```python
from build123d import *

# Parameters (mm, degrees)
BASE_BLOCK_SKETCH_W       = 50
BASE_BLOCK_SKETCH_H       = 30
BASE_BLOCK_50X30X25_DEPTH = 25
CORNER_STEP_5MM_DEPTH     = 5
LOWER_PLATE_SKETCH_W      = 19.888158271
LOWER_PLATE_SKETCH_H      = 16.417205811
LOWER_PLATE_5MM_DEPTH     = 5
LEG_SKETCH_W              = 5
LEG_SKETCH_H              = 16.417205811
LEG_15MM_DEPTH            = 15
TAPERED_WEB_16_5MM_DEPTH  = 16.5


with BuildPart() as part:
    # Base Block Sketch → Base Block 50x30x25 (new body)
    with BuildSketch(Plane(origin=(0, 0, 0), x_dir=(1, 0, 0), z_dir=(0, 1, 0))):
        with Locations((25, 15)):
            Rectangle(BASE_BLOCK_SKETCH_W, BASE_BLOCK_SKETCH_H)
    extrude(amount=BASE_BLOCK_50X30X25_DEPTH)

    # Corner Step Sketch → Corner Step 5mm (add)
    with BuildSketch(Plane(origin=(0, 0, 0), x_dir=(1, 0, 0), z_dir=(0, 1, 0))):
        Polygon((0, 30), (0, 40), (10, 40), (10, 35), (40, 35), (40, 40), (50, 40), (50, 30), (50, 0), (0, 0), align=None)
    extrude(amount=CORNER_STEP_5MM_DEPTH)

    # Lower Plate Sketch → Lower Plate 5mm (add)
    with BuildSketch(Plane.XZ):
        Polygon((6.770734002, 0), (0, 0), (0, -16.417205811), (6.770734002, -16.417205811), (20.078313967, -16.417205811), (20.078313967, 0), align=None)
        with Locations((40.055920865, -8.208602906)):
            Rectangle(LOWER_PLATE_SKETCH_W, LOWER_PLATE_SKETCH_H)
    extrude(amount=LOWER_PLATE_5MM_DEPTH)

    # Leg Sketch → Leg 15mm (add)
    with BuildSketch(Plane(origin=(0, -5, 0), x_dir=(-1, 0, 0), z_dir=(0, -1, 0))):
        with Locations((-2.5, 8.208602906)):
            Rectangle(LEG_SKETCH_W, LEG_SKETCH_H)
        with Locations((-47.5, 8.208602906)):
            Rectangle(LEG_SKETCH_W, LEG_SKETCH_H)
    extrude(amount=LEG_15MM_DEPTH)

    # Tapered Web Sketch → Tapered Web 16.5mm (add)
    with BuildSketch(Plane.XY):
        Polygon((30.111841729, -5), (45, -20), (45, -5), align=None)
        Polygon((5, -5), (5, -20), (20, -5), align=None)
    extrude(amount=-TAPERED_WEB_16_5MM_DEPTH)


solid = part.part
```
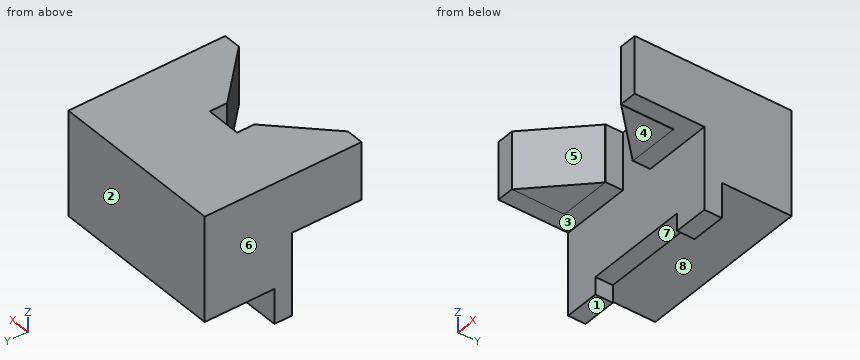
Input: part model. Units: mm. Frame: model coordinates. Face numbers are marked on the shaded views. A direction names the side the tool comes from. Give positions to 0.01 mm unless a question says otherwise; leave off trailing zeros. Write each loop counter-clockwise with the first axis right and the second up, starting at its lowest first coordinate (ties: lowest second). Pieces come first, ordered by that corner, then holes. Notation, with made-up numbers: (-12.75, 21.5) - (46.25, 21.5) arc R7 ccw to (46.25, 28.5) - close; hole circle Ø3 at (-7, -25.5). An arc over 180 degrees is marked (long way). Write item = value, one per line. Start each with the question number.
1. Section query C-C, the plane z = -10. Output: boundary loops of the cut face in (x, y).
2. Section query B-B, the plane x = 12. Output: boundary loops of the cut face in (y, z), then the cut area to 3 significant figures.
3. Section query D-D, the plane y = -6. Output: boundary loops of the cut face in (x, z), then the cut area to 3 significant figures.
4. Ray query, L1, parallel to Y at x = 10, z = -27; L2, parallel to Z at x = 13, y = 9.5; L3, parallel to Z at x = 41, y = -13. Return the intervals inside material, ascending.
5. Section query A-A, the plane y = -12. Output: boundary loops of the cut face in (x, z).
6. First-contact query: pin 1 Ø6 at (x, y) = (33, 19) entering from -Z; pin 2 Ø3 at (x, z) = (7.5, -33.5) entering from -Y; pin 3 Ø5 at (y, z) = (-14.5, -16.5) entering from -X; pin 4 Ø2 at (x, z) = (42, -4.5) entering from -Y (3 decimals). Flat tips, straight axial feed; report the tip coordinate or a pass-through.
7. Mould query, pull axis Y, two halves, no side actions, for the marked faces 1, 2 and 3. Classes: released by +Y, released by -Y, zero draft, split by the parting line, or undercut.
8. Access query for the marked faces 4, 5, 6, 7 and 8. Directions: +Z, -Z, +X, -X, +Y, -Y. A direction counts if a zero-diameter tool reaches every point of the face in a straight line with its end or side. Return the directions, or none.
Check sheet entries:
q1.outline = (0, -20) - (5, -20) - (20, -5) - (20.08, -5) - (20.08, 0) - (30.11, 0) - (30.11, -5) - (45, -20) - (50, -20) - (50, 25) - (0, 25) - close
q2.outline = (-13, -16.5) - (-5, -16.5) - (-5, -16.42) - (0, -16.42) - (0, -35) - (5, -35) - (5, -30) - (25, -30) - (25, 0) - (-13, 0) - close
q2.area = 989 mm2
q3.outline = (0, -16.42) - (5, -16.42) - (5, -16.5) - (19, -16.5) - (19, 0) - (0, 0) - close; (31.1, -16.5) - (45, -16.5) - (45, -16.42) - (50, -16.42) - (50, 0) - (31.1, 0) - close
q3.area = 624 mm2
q4.L1 = 0 to 25
q4.L2 = -30 to 0
q4.L3 = -16.5 to 0
q5.outline = (0, -16.42) - (5, -16.42) - (5, -16.5) - (13, -16.5) - (13, 0) - (0, 0) - close; (37.06, -16.5) - (45, -16.5) - (45, -16.42) - (50, -16.42) - (50, 0) - (37.06, 0) - close
q6.pin_1 = -30
q6.pin_2 = 0
q6.pin_3 = 0
q6.pin_4 = -17.985
q7.face_1 = zero draft
q7.face_2 = released by +Y
q7.face_3 = undercut
q8.face_4 = -Z, +X, -X, -Y
q8.face_5 = +Z, -Z, -Y
q8.face_6 = +Z, -Z, -X, +Y, -Y
q8.face_7 = -Z, +Y, -Y
q8.face_8 = -Z, +X, -X, +Y
